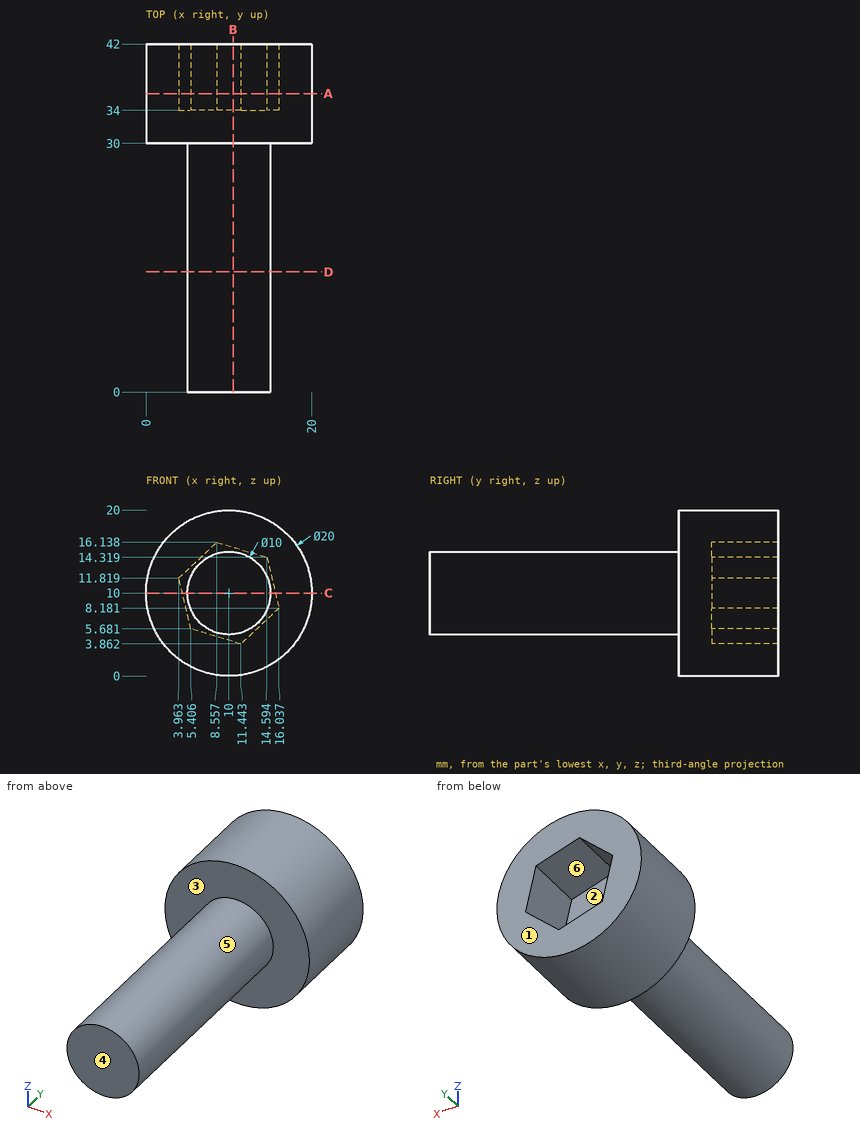
Part print with two shaded views. Sizes in mm from the minimum x, y, z corner. A direction names the side the tool comes from. Round coordinates to 2 decimals unless told otherwise and drop trailing zeros. Order: outer loops, then holes, each group sorted by start corner. A loop starts at its lowest first (then second) coordinate and runs counter-clockwise, first axis right, second up. Notation, with made-up numbers: (48.25, -4) - (65.25, -4) arc R17 ccw to (65.25, 28) - close; hole circle Ø5 at (-14, 87). An arc over 180 degrees is marked (long way). Answer in a Markdown table with one row per item. Add a question column.
(1) Band-saw the part on C-C on z = 10. List the corners of the cut face in (x, y), and give its area (3 significant figures).
(2) Mould opens along Z. For the marked faces 4, 5 and 6 say: +Z half, -Z half, draft (parallel to the pull), parting line (faces both ways), or undercut.
(3) Drop flat-ended pins along their axis: pin 1 Ø3 at (y, z) = (25, 5.5) entering from -X; pin 2 Ø8 at (x, y) = (8.5, 18.5) entering from -Z; pin 3 Ø3 at (x, y) = (17.5, 31) entering from +Z. Give the stop position or say it passes through.
(4) Band-saw the part on D-D on y = 14.5. List the corners of the cut face in (x, z).
(5) 3-axis set-ups, long thin cutter, end or side, ignore diameter. For the marked faces 1, 2 and 3: which of +Z, -Z, +X, -X, +Y, -Y reach the whole face in a straight line?
(6) Probe L1, parallel to Y at x = 3.5, z = 5.75; L2, parallel to X at y = 37, z = 7.5 (1 decimal); L3, parallel to X at y = 39, z = 5.75. List the from-to ranges inside material, lowest first. Write a range as [from, to].
(7) Band-saw the part on A-A on y = 36. List the corners of the cut face in (x, z), and give its area (3 significant figures).
(8) Band-saw the part on B-B on x = 10.5. List the corners of the cut face in (y, z) (1 decimal).
Data:
| question | item | result |
|---|---|---|
| 1 | outline | (0, 30) - (5, 30) - (5, 0) - (15, 0) - (15, 30) - (20, 30) - (20, 42) - (15.61, 42) - (15.61, 34) - (4.39, 34) - (4.39, 42) - (0, 42) - close |
| 1 | area | 450 mm^2 |
| 2 | face 4 | draft |
| 2 | face 5 | parting line |
| 2 | face 6 | undercut |
| 3 | pin 1 | stops at x = 6 |
| 3 | pin 2 | stops at z = 5 |
| 3 | pin 3 | stops at z = 18 |
| 4 | outline | circle Ø10 at (10, 10) |
| 5 | face 1 | +Z, -Z, +X, -X, +Y |
| 5 | face 2 | +Y |
| 5 | face 3 | -Y |
| 6 | L1 | y = [30, 42] |
| 6 | L2 | x = [0.3, 5], [15.3, 19.7] |
| 6 | L3 | x = [0.95, 5.39], [13.45, 19.05] |
| 7 | outline | circle Ø20 at (10, 10); hole (3.96, 11.82) - (5.41, 5.68) - (11.44, 3.86) - (16.04, 8.18) - (14.59, 14.32) - (8.56, 16.14) - close |
| 7 | area | 211 mm^2 |
| 8 | outline | (0, 5) - (30, 5) - (30, 0) - (42, 0) - (42, 4.1) - (34, 4.1) - (34, 15.6) - (42, 15.6) - (42, 20) - (30, 20) - (30, 15) - (0, 15) - close |
